from build123d import *

# Parameters (mm, degrees)
SKETCH1_R               = 11
SKETCH1_R_2             = 2
BOSS_EXTRUDE1_DEPTH     = 2
SKETCH2_R               = 4.5
BOSS_EXTRUDE2_DEPTH     = 4
CUT_EXTRUDE1_DEPTH      = 17.673332001
CUT_EXTRUDE1_DEPTH_BACK = 17.673332001
SKETCH3_R               = 2


with BuildPart() as part:
    # Sketch1 → Boss-Extrude1 (new body)
    with BuildSketch(Plane(origin=(0, 0, 0), x_dir=(1, 0, 0), z_dir=(0, 1, 0))):
        with Locations(Location((0, 0, 0), (0, 0, 270))):
            Circle(SKETCH1_R)
        with Locations(Location((0, 7.5, 0), (0, 0, 270))):
            Circle(SKETCH1_R_2, mode=Mode.SUBTRACT)
        with Locations(Location((7.5, 0, 0), (0, 0, 270))):
            Circle(SKETCH1_R_2, mode=Mode.SUBTRACT)
        with Locations(Location((0, -7.5, 0), (0, 0, 270))):
            Circle(SKETCH1_R_2, mode=Mode.SUBTRACT)
        with Locations(Location((-7.5, 0, 0), (0, 0, 270))):
            Circle(SKETCH1_R_2, mode=Mode.SUBTRACT)
    extrude(amount=BOSS_EXTRUDE1_DEPTH)

    # Sketch2 → Boss-Extrude2 (add)
    with BuildSketch(Plane(origin=(0, 2, 0), x_dir=(1, 0, 0), z_dir=(0, 1, 0))):
        with Locations(Location((0, 0, 0), (0, 0, 270))):
            Circle(SKETCH2_R)
    extrude(amount=BOSS_EXTRUDE2_DEPTH)

    # Sketch3 → Cut-Extrude1 (cut, two sides: drawn at the far end of the back side and taken through both)
    with BuildSketch(Plane(origin=(0, 6, 0), x_dir=(1, 0, 0), z_dir=(0, 1, 0)).offset(-CUT_EXTRUDE1_DEPTH_BACK)):
        with Locations(Location((0, 0, 0), (0, 0, 270))):
            Circle(SKETCH3_R)
    extrude(amount=CUT_EXTRUDE1_DEPTH + CUT_EXTRUDE1_DEPTH_BACK, mode=Mode.SUBTRACT)


solid = part.part
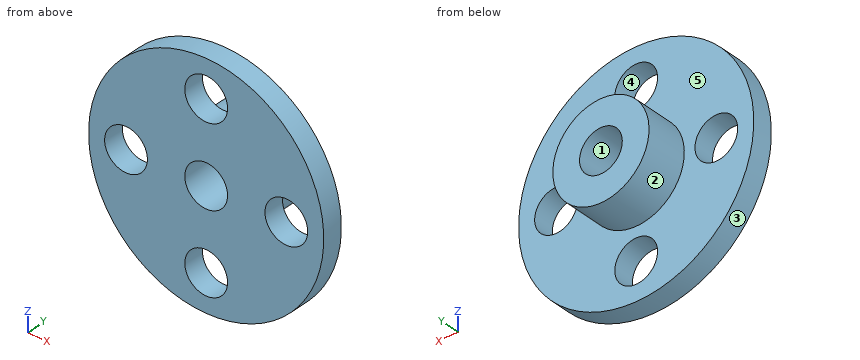
Geometry: final body of the model. Coordinates: model frame, mm. Face numbers are marked on the shaded views. A direction names the side the tool comes from. Round coordinates to 2 decimals unless told otherwise and drop trailing zeros. Loops run counter-clockwise (first coordinate to the right, second up) from the corner with the lowest first, then second, coordinate; pieces in that order, holes last. Notation, with made-up numbers: M 73.25,5.25 L 80.25,5.25 A6 ccw 80.25,13.25 Z; hole C -11,5.25 d4. An arc over 180 degrees is marked long. One line per question, with ' | ' between items.
(1) Cut plane C-C on y = 1.4. Return the cut outline in (x, z).
Check result:
outline: C 0,0 d22; hole C -7.5,0 d4; hole C 0,-7.5 d4; hole C 0,0 d4; hole C 0,7.5 d4; hole C 7.5,0 d4
(2) Cut plane D-D on x = 7.5. Return the cut outline in (y, z).
Check result:
outline: M 0,-8.05 L 2,-8.05 L 2,-2 L 0,-2 Z; M 0,2 L 2,2 L 2,8.05 L 0,8.05 Z
(3) Cut plane B-B on z = -7.75. Return the cut outline in (x, y), plus the area to 3 significant figures.
Check result:
outline: M -7.81,0 L -1.98,0 L -1.98,2 L -7.81,2 Z; M 1.98,0 L 7.81,0 L 7.81,2 L 1.98,2 Z | area: 23.3 mm2
(4) Cut plane A-A on x = 0. Return the cut outline in (y, z), plus the area to 3 significant figures.
Check result:
outline: M 0,-11 L 2,-11 L 2,-9.5 L 0,-9.5 Z; M 0,-5.5 L 2,-5.5 L 2,-4.5 L 6,-4.5 L 6,-2 L 0,-2 Z; M 0,2 L 6,2 L 6,4.5 L 2,4.5 L 2,5.5 L 0,5.5 Z; M 0,9.5 L 2,9.5 L 2,11 L 0,11 Z | area: 40.0 mm2
(5) Material intervals for line 1 along X through (y, z) = (1.5, 0); line 2 along X through (y, z) = (0.8, 0.75); line 3 along Y through (x, z) = (-8.75, -5), sorted ascending. Write a range as from..to.
Check result:
line 1: x = -11..-9.5, -5.5..-2, 2..5.5, 9.5..11 | line 2: x = -10.97..-9.35, -5.65..-1.85, 1.85..5.65, 9.35..10.97 | line 3: y = 0..2
(6) Access query for the marked faces 1 and 2. Directions: +Z, -Z, +X, -X, +Y, -Y. A direction counts if a zero-diameter tool reaches every point of the face in a straight line with its end or side. Return the directions, or none.
Check result:
face 1: +Y, -Y | face 2: +Y
(7) Contact query for flat-ended pins moving along their axis: P1, Ø6, axis at x = -6, z = 5.5, coming from the +Y side; P2, Ø3.5, axis at x = -7.5, z = 0, coming from the -Y side; P3, Ø2, axis at y = 2, z = -1.5, coming from the +X side; P4, Ø1, axis at x = -3.5, y = 3.5, coming from the +Z side. Output: stop coordinate, or through.
Check result:
P1: stops at y = 2 | P2: passes through | P3: stops at x = 10.99 | P4: stops at z = 3.35
(8) Pull-direction query (X, two-part tool) for the marked faces 3, 4 and 5; classes: +X half, -X half, draft (parallel to the pull), parting line (faces both ways), or undercut.
Check result:
face 3: parting line | face 4: undercut | face 5: draft
